The model under review builds one solid part; all positions refer to its coordinate system, in mm. A direction names the side the tool comes from. Coordinates: 2 decimals unless noted, no trailing zeros. Write each loop counter-clockwise with the first axis right and the second up, starting at its lowest first coordinate (ties: lowest second). Pieces come first, ordered by that corner, then holes.
```python
from build123d import *

# Parameters (mm, degrees)
SKETCH1_R           = 64
BOSS_EXTRUDE1_DEPTH = 25
SKETCH2_R           = 70
CUT_EXTRUDE1_DEPTH  = 41.5
CHAMFER1_SIZE       = 2
FILLET1_R           = 2
CUT_EXTRUDE2_DEPTH  = 41.5
BOSS_EXTRUDE2_START = -50
BOSS_EXTRUDE2_DEPTH = 50
CHAMFER2_SIZE       = 10


with BuildPart() as part:
    # Sketch1 → Boss-Extrude1 (new, symmetric)
    with BuildSketch(Plane(origin=(0, 0, 0), x_dir=(1, 0, 0), z_dir=(0, 1, 0))):
        with BuildLine():
            Line((-172, 0), (172, 0))
            Line((172, 0), (172, 30))
            Line((172, 30), (112, 30))
            Line((112, 30), (91.468409221, 116.66864358))
            ThreePointArc((91.468409221, 116.66864358), (0, 189), (-91.468409221, 116.66864358))
            Line((-91.468409221, 116.66864358), (-112, 30))
            Line((-112, 30), (-172, 30))
            Line((-172, 30), (-172, 0))
        make_face()
        with Locations(Location((0, 95, 0), (0, 0, 270))):
            Circle(SKETCH1_R, mode=Mode.SUBTRACT)
    extrude(amount=BOSS_EXTRUDE1_DEPTH, both=True)

    # Sketch2 → Cut-Extrude1 (cut)
    with BuildSketch(Plane.XZ.offset(25)):
        with Locations(Location((0, -95, 0), (0, 0, 270))):
            Circle(SKETCH2_R)
    extrude(amount=-CUT_EXTRUDE1_DEPTH, mode=Mode.SUBTRACT)

    # Chamfer1
    chamfer1_edges = [part.edges().sort_by_distance(p)[0] for p in [
        (0, -25, -25),
    ]]
    chamfer(chamfer1_edges, length=CHAMFER1_SIZE)

    # Fillet1
    fillet1_edges = [part.edges().sort_by_distance(p)[0] for p in [
        (0, 16.5, -25),
    ]]
    fillet(fillet1_edges, radius=FILLET1_R)

    # Sketch3 → Cut-Extrude2 (cut)
    with BuildSketch(Plane(origin=(0, 0, -30), x_dir=(-1, 0, 0), z_dir=(0, 0, -1))):
        with BuildLine():
            Line((135, 11), (145, 11))
            ThreePointArc((145, 11), (156, 0), (145, -11))
            Line((145, -11), (135, -11))
            ThreePointArc((135, -11), (124, 0), (135, 11))
        make_face()
        with BuildLine():
            Line((-145, 11), (-135, 11))
            ThreePointArc((-135, 11), (-124, 0), (-135, -11))
            Line((-135, -11), (-145, -11))
            ThreePointArc((-145, -11), (-156, 0), (-145, 11))
        make_face()
    extrude(amount=-CUT_EXTRUDE2_DEPTH, mode=Mode.SUBTRACT)

    # Sketch4 → Boss-Extrude2 (add)
    with BuildSketch(Plane.XZ.offset(25).offset(BOSS_EXTRUDE2_START)):
        with BuildLine():
            Line((-112, -30), (-112, -190))
            Line((-112, -190), (112, -190))
            Line((112, -190), (112, -30))
            Line((112, -30), (91.468409221, -116.66864358))
            ThreePointArc((91.468409221, -116.66864358), (0, -189), (-91.468409221, -116.66864358))
            Line((-91.468409221, -116.66864358), (-112, -30))
        make_face()
    extrude(amount=BOSS_EXTRUDE2_DEPTH)

    # Chamfer2
    chamfer2_edges = [part.edges().sort_by_distance(p)[0] for p in [
        (112, 0, -190),
        (-112, 0, -190),
    ]]
    chamfer(chamfer2_edges, length=CHAMFER2_SIZE)


solid = part.part
```
Item 1: For pin 1 (5 mm diameter, centred on y = -4.5, z = -168.5, fed in from +X); pin 2 (2 mm diameter, centred on y = 7.5, z = -104, fed in from -X), all flat-tipped, find the tip position at first contact; note any pin that passes through.
Solved:
pin 1: stops at x = 112
pin 2: stops at x = -112
Item 2: To check wall thickness, follow line 1 along X through (y, z) = (2, -95); line 2 along X through (y, z) = (19.75, -95); line 3 along Z through (x, y) = (-122.5, 14.5). State the ranges of each line that lie inside material, in increasing order.
Solved:
line 1: x = -112 to -70, 70 to 112
line 2: x = -112 to -64, 64 to 112
line 3: z = -30 to 0
Item 3: Take a section at A-A, the plane y = 0. Write out the cut boundary in (x, z), plus the area to 3 significant figures.
Solved:
outline: (-172, -30) - (-156, -30) - (-156, 0) - (-172, 0) - close; (-124, -30) - (-112, -30) - (-112, -180) - (-102, -190) - (102, -190) - (112, -180) - (112, -30) - (124, -30) - (124, 0) - (-124, 0) - close; (156, -30) - (172, -30) - (172, 0) - (156, 0) - close; hole circle Ø140 at (0, -95)
area: 28,700 mm2
Item 4: Take a section at B-B, the plane x = 0. Write out the cut boundary in (y, z).
Solved:
outline: (-25, -190) - (25, -190) - (25, -159) - (16.5, -159) - (16.5, -163) arc R2 cw to (14.5, -165) - (-23, -165) - (-25, -167) - close; (-25, -23) - (-23, -25) - (14.5, -25) arc R2 cw to (16.5, -27) - (16.5, -31) - (25, -31) - (25, 0) - (-25, 0) - close
Item 5: Machinability: for faces 4 (the face through (46, 16.5, -140)), 5 (the face through (142.4, 11.5, -30)), 6 (the face through (140, -11, -15)), which of the approach directions +Z, -Z, +X, -X, +Y, -Y give a long, thin tool a straight path to every point of the face, cutting with its end or side? Answer none if there is none.
Solved:
face 4: -Y
face 5: -Z, +X, +Y, -Y
face 6: +Z, -Z
Item 6: Mouldability with a two-part tool opening along Y and no side actions: class faces 1 (the face through (124, 0, -15)), 2 (the face through (-2, 25, -30)), 3 (the face through (-42.594, -4.512, -39.45)) as pulls with the +Y half, pulls with the -Y half, needs draft (parallel to the pull), parting line crosses it, or undercut.
Solved:
face 1: undercut
face 2: pulls with the +Y half
face 3: needs draft
Item 7: Take a section at C-C, the plane z = -95. Write out the cut boundary in (x, y), plus the area to 3 significant figures.
Solved:
outline: (-112, -25) - (-72, -25) - (-70, -23) - (-70, 14.5) arc R2 cw to (-68, 16.5) - (-64, 16.5) - (-64, 25) - (-112, 25) - close; (64, 16.5) - (68, 16.5) arc R2 cw to (70, 14.5) - (70, -23) - (72, -25) - (112, -25) - (112, 25) - (64, 25) - close
area: 4,300 mm2
